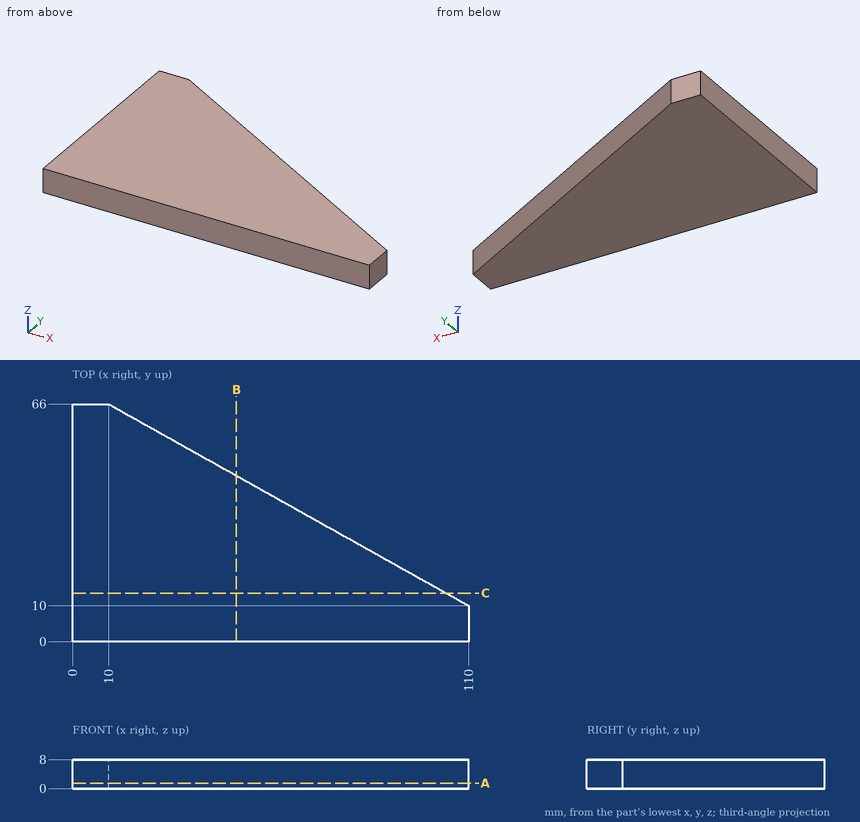
Source: three-view drawing plus pictorial views. Frame: mm from the lowest corner of the part. Round coordinates to 2 decimals unless told otherwise and drop trailing zeros. Order: outer loops, then holes, each group sorted by start corner. A loop starts at its lowest first (then second) coordinate and runs counter-clockwise, first axis right, second up. Notation, with made-up numbers: (9.25, -37.5) -> (31.25, -37.5) arc R17 cw to (31.25, -21.5) -> close; hole circle Ø4 at (-37.75, -27). An arc over 180 degrees is marked (long way). Use one line per item in the form item = value.
(1) Section C-C on y = 13.5. Return loops of the section in (x, z).
Results list:
outline = (0, 0) -> (103.75, 0) -> (103.75, 8) -> (0, 8) -> close
(2) Section A-A on z = 1.5. Return loops of the section in (x, y).
Results list:
outline = (0, 0) -> (110, 0) -> (110, 10) -> (10, 66) -> (0, 66) -> close
(3) Section B-B on x = 45.5. Return loops of the section in (y, z).
Results list:
outline = (0, 0) -> (46.12, 0) -> (46.12, 8) -> (0, 8) -> close
(4) Ray query, probe 1 along Y at (x, z) = (37.5, 0.5); probe 2 along Y at (x, z) = (15.5, 0.5); probe 3 along X at (y, z) = (57, 0.5). Return the intervals inside material, ascending. Write a range as [from, to].
Results list:
probe_1 = [0, 50.6]
probe_2 = [0, 62.92]
probe_3 = [0, 26.07]
(5) First-contact query: pin 1 Ø1 at (y, z) = (35.5, 7) entering from +X. Flat tip, straight axial feed; report the tip coordinate or a pass-through.
Results list:
pin_1 = 65.36
